For this review, use the dimensioned drawing (mm, ordinates from the lowest corner) and the shaded views. A direction names the side the tool comes from. Give positions to 0.01 mm unless a question says otherwise; leave off trailing zeros. Order: outer loops, then holes, each group sorted by start corner. A loop starts at its lowest first (then second) coordinate and runs counter-clockwise, first axis right, second up. Notation, with made-up numbers: (-27, 84) - (-23, 84) arc R25 cw to (-23, 108) - close; hole circle Ø3 at (20, -36). An arc over 180 degrees is marked (long way). One line per item, written item: value.
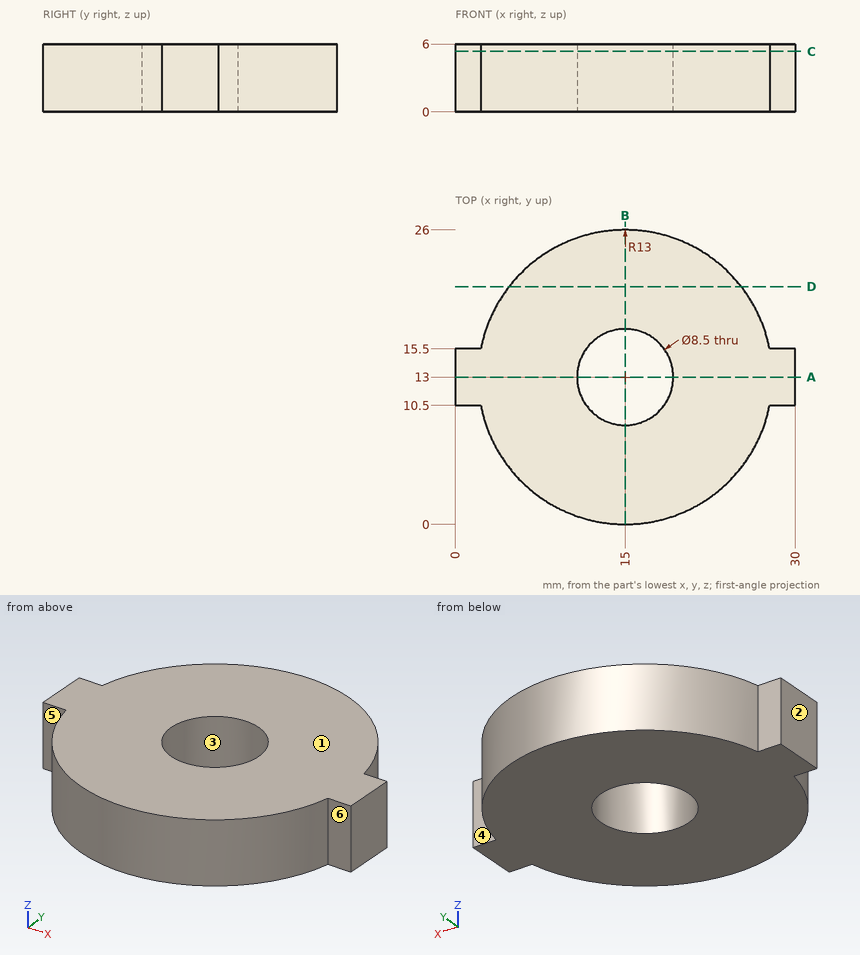
(1) Machinability: for the marked faces 4, 5 and 6, which of the approach directions +Z, -Z, +X, -X, +Y, -Y give a long, thin tool a straight path to every point of the face, cutting with its end or side? Answer none if there is none.
Answers below:
face 4: +Z, -Z, +X, +Y
face 5: +Z, -Z, -X, -Y
face 6: +Z, -Z, +X, -Y
(2) Wall thickness on line 1 (X direction, y = 13, z = 4.4); line 2 (X direction, y = 11, z = 3); line 3 (Y direction, x = 14.5, z = 2.15): over which ranges is each line inside the solid? List them lowest first. Write a range as from..to.
Answers below:
line 1: x = 0..10.75, 19.25..30
line 2: x = 0..11.25, 18.75..30
line 3: y = 0.01..8.78, 17.22..25.99
(3) For P1, Ø1.5, axis at x = 17, z = 2, coming from the -Y side; P2, Ø1.1, axis at x = 29, z = 2.5, coming from the -Y side; P3, Ø3, axis at x = 7, z = 4, coming from the +Y side, all flat-tipped, find the tip position at first contact; note any pin that passes through.
Answers below:
P1: stops at y = 0.06
P2: stops at y = 10.5
P3: stops at y = 24.26
(4) Take a section at C-C (z = 5.35). Write out the cut boundary in (x, y).
Answers below:
outline: (0, 10.5) - (2.24, 10.5) arc R13 ccw to (27.76, 10.5) - (30, 10.5) - (30, 15.5) - (27.76, 15.5) arc R13 ccw to (2.24, 15.5) - (0, 15.5) - close; hole circle Ø8.5 at (15, 13)
(5) Draft analysis for pull direction X (two halves, no side actions). For the marked faces 1, 2 and 3, state which applies: pulls with the +X half, pulls with the -X half, needs draft (parallel to the pull), parting line crosses it, or undercut.
Answers below:
face 1: needs draft
face 2: pulls with the -X half
face 3: undercut
(6) Take a section at D-D (y = 21). Write out the cut boundary in (x, z), then the cut area to 3 significant figures.
Answers below:
outline: (4.75, 0) - (25.25, 0) - (25.25, 6) - (4.75, 6) - close
area: 123 mm^2
(7) Take a section at B-B (x = 15). Write out the cut boundary in (y, z), then the cut area to 3 significant figures.
Answers below:
outline: (0, 0) - (8.75, 0) - (8.75, 6) - (0, 6) - close; (17.25, 0) - (26, 0) - (26, 6) - (17.25, 6) - close
area: 105 mm^2
(8) Take a section at A-A (y = 13). Write out the cut boundary in (x, z), then the cut area to 3 significant figures.
Answers below:
outline: (0, 0) - (10.75, 0) - (10.75, 6) - (0, 6) - close; (19.25, 0) - (30, 0) - (30, 6) - (19.25, 6) - close
area: 129 mm^2
